Geometry check sheet. Reference: the model listing, model coordinates, mm. Face numbers are marked on the shaded views. A direction names the side the tool comes from. Round coordinates to 2 decimals unless told otherwise and drop trailing zeros. Order: outer loops, then holes, each group sorted by start corner. A loop starts at its lowest first (then second) coordinate and runs counter-clockwise, first axis right, second up. Notation, with made-up numbers: (54, 19) -> (60, 19) arc R8 ccw to (60, 31) -> close; hole circle Ø6 at (14, 44). An arc over 180 degrees is marked (long way). Use a Markdown table: item, result. Add a question column.
Item 1: Set-up check for the marked faces 1, 2, 3 and 4: record each of +Z, -Z, +X, -X, +Y, -Y from which the full face is reachable in a straight line by a thin tool's end or side.
Item 2: Sectioned sample at D-D, the plane y = 27. Record the cut outline in (x, z), and give its area (3 significant figures).
Item 3: Gauge pin test, flat ends, axial feed: pin 1 Ø5 at (y, z) = (8.5, -57) entering from -X; pin 2 Ø5 at (y, z) = (11, -56) entering from +X; pin 3 Ø10 at (x, z) = (-5, 64.5) entering from -Y. Record the tip position at first contact, or that the pin passes through.
Item 4: Sectioned sample at C-C, the plane z = 0. Record the cut outline in (x, y).
Item 5: Sectioned sample at A-A, the plane y = 7. Record the cut outline in (x, z) (1 decimal).
Item 6: Sectioned sample at B-B, the plane x = 0. Record the cut outline in (y, z).
Item 7: Mould release check, pull along Z, two halves, no side actions. Record for the marked faces 5, 6 and 7: pulls with the +Z half, pulls with the -Z half, needs draft (parallel to the pull), parting line crosses it, or undercut.
Item 8: Material ranges on probe 1 along Y at (x, z) = (-38, 44); probe 2 along Y at (x, z) = (24, 11); probe 3 along X at (y, z) = (21.25, 0), recorded low to high. Write a range as [from, to].
from build123d import *

# Parameters (mm, degrees)
BASE_DISC_20MM_DEPTH        = 20
THREE_LOBE_BOSS_15MM_DEPTH  = 15
COUNTERBORE_PROFILE_R       = 30
COUNTERBORE_20MM_DEEP_DEPTH = 20
THROUGH_BORE_PROFILE_R      = 15
THROUGH_BORE_DEPTH          = 107.05840812


with BuildPart() as part:
    # Base Disc Profile → Base Disc 20mm (new body)
    with BuildSketch(Plane(origin=(0, 0, 0), x_dir=(1, 0, 0), z_dir=(0, 1, 0))):
        with BuildLine():
            Line((-20, 53.37602458), (-20, 59.741108125))
            ThreePointArc((-20, 59.741108125), (0, 63), (20, 59.741108125))
            Line((20, 59.741108125), (20, 53.37602458))
            ThreePointArc((20, 53.37602458), (49.363448016, 28.5), (56.22499324, -9.367504214))
            Line((56.22499324, -9.367504214), (61.737317286, -12.550045987))
            ThreePointArc((61.737317286, -12.550045987), (54.559600438, -31.5), (41.737317286, -47.191062138))
            Line((41.737317286, -47.191062138), (36.22499324, -44.008520366))
            ThreePointArc((36.22499324, -44.008520366), (0, -57), (-36.22499324, -44.008520366))
            Line((-36.22499324, -44.008520366), (-41.737317286, -47.191062138))
            ThreePointArc((-41.737317286, -47.191062138), (-54.559600438, -31.5), (-61.737317286, -12.550045987))
            Line((-61.737317286, -12.550045987), (-56.22499324, -9.367504214))
            ThreePointArc((-56.22499324, -9.367504214), (-49.363448016, 28.5), (-20, 53.37602458))
        make_face()
    extrude(amount=BASE_DISC_20MM_DEPTH)

    # Three-Lobe Profile → Three-Lobe Boss 15mm (add)
    with BuildSketch(Plane(origin=(0, 20, 0), x_dir=(1, 0, 0), z_dir=(0, 1, 0))):
        with BuildLine():
            ThreePointArc((39.473039737, 41.120300752), (0, 33), (-39.473039737, 41.120300752))
            ThreePointArc((-39.473039737, 41.120300752), (-49.363448016, 28.5), (-55.347744931, 13.624504801))
            ThreePointArc((-55.347744931, 13.624504801), (-28.578838325, -16.5), (-15.874705194, -54.744805553))
            ThreePointArc((-15.874705194, -54.744805553), (-1.422355425, -56.98225079), (13.123625771, -55.468643815))
            ThreePointArc((13.123625771, -55.468643815), (27.648504036, -17.766556361), (55.906633869, 11.110728574))
            ThreePointArc((55.906633869, 11.110728574), (49.994641111, 27.377652568), (39.473039737, 41.120300752))
        make_face()
        with BuildLine():
            ThreePointArc((-39.473039737, 41.120300752), (-44.717521746, 43.555362101), (-49.812494678, 46.289473684))
            ThreePointArc((-49.812494678, 46.289473684), (-58.889727457, 34), (-64.994107477, 19.994148975))
            ThreePointArc((-64.994107477, 19.994148975), (-60.078810924, 16.948828776), (-55.347744931, 13.624504801))
            ThreePointArc((-55.347744931, 13.624504801), (-49.363448016, 28.5), (-39.473039737, 41.120300752))
        make_face()
        with BuildLine():
            ThreePointArc((-49.812494678, 46.289473684), (-52.867031225, 48.117274965), (-55.854579687, 50.052631579))
            ThreePointArc((-55.854579687, 50.052631579), (-64.951905284, 37.5), (-71.274140317, 23.345169137))
            ThreePointArc((-71.274140317, 23.345169137), (-68.104298093, 21.725554581), (-64.994107477, 19.994148975))
            ThreePointArc((-64.994107477, 19.994148975), (-58.889727457, 34), (-49.812494678, 46.289473684))
        make_face()
        with BuildLine():
            ThreePointArc((13.123625771, -55.468643815), (-1.422355425, -56.98225079), (-15.874705194, -54.744805553))
            ThreePointArc((-15.874705194, -54.744805553), (-15.361289177, -60.504190877), (-15.181612799, -66.283622659))
            ThreePointArc((-15.181612799, -66.283622659), (-1.676596285, -67.979327923), (11.895593178, -66.951436601))
            ThreePointArc((11.895593178, -66.951436601), (12.343713059, -61.192298339), (13.123625771, -55.468643815))
        make_face()
        with BuildLine():
            ThreePointArc((11.895593178, -66.951436601), (-1.676596285, -67.979327923), (-15.181612799, -66.283622659))
            ThreePointArc((-15.181612799, -66.283622659), (-15.237266868, -69.842829546), (-15.41956063, -73.397800716))
            ThreePointArc((-15.41956063, -73.397800716), (-1.839450143, -74.977439428), (11.801783935, -74.065632354))
            ThreePointArc((11.801783935, -74.065632354), (11.7853983, -70.507699919), (11.895593178, -66.951436601))
        make_face()
        with BuildLine():
            ThreePointArc((49.812494678, 46.289473684), (44.717521746, 43.555362101), (39.473039737, 41.120300752))
            ThreePointArc((39.473039737, 41.120300752), (49.994641111, 27.377652568), (55.906633869, 11.110728574))
            ThreePointArc((55.906633869, 11.110728574), (60.78874038, 14.198368606), (65.840986006, 16.998957666))
            ThreePointArc((65.840986006, 16.998957666), (59.652455781, 32.643292102), (49.812494678, 46.289473684))
        make_face()
        with BuildLine():
            ThreePointArc((55.854579687, 50.052631579), (52.867031225, 48.117274965), (49.812494678, 46.289473684))
            ThreePointArc((49.812494678, 46.289473684), (59.652455781, 32.643292102), (65.840986006, 16.998957666))
            ThreePointArc((65.840986006, 16.998957666), (69.029934048, 18.576855661), (72.272995877, 20.04031105))
            ThreePointArc((72.272995877, 20.04031105), (65.797824819, 35.995086458), (55.854579687, 50.052631579))
        make_face()
    extrude(amount=THREE_LOBE_BOSS_15MM_DEPTH)

    # Counterbore Profile → Counterbore 20mm Deep (cut)
    with BuildSketch(Plane(origin=(0, 35, 0), x_dir=(1, 0, 0), z_dir=(0, 1, 0))):
        with Locations(Location((0, 0, 0), (0, 0, 270))):
            Circle(COUNTERBORE_PROFILE_R)
    extrude(amount=-COUNTERBORE_20MM_DEEP_DEPTH, mode=Mode.SUBTRACT)

    # Through Bore Profile → Through Bore (cut, through all)
    with BuildSketch(Plane(origin=(0, 15, 0), x_dir=(1, 0, 0), z_dir=(0, 1, 0))):
        with Locations(Location((0, 0, 0), (0, 0, 270))):
            Circle(THROUGH_BORE_PROFILE_R)
    extrude(amount=-THROUGH_BORE_DEPTH, mode=Mode.SUBTRACT)


solid = part.part
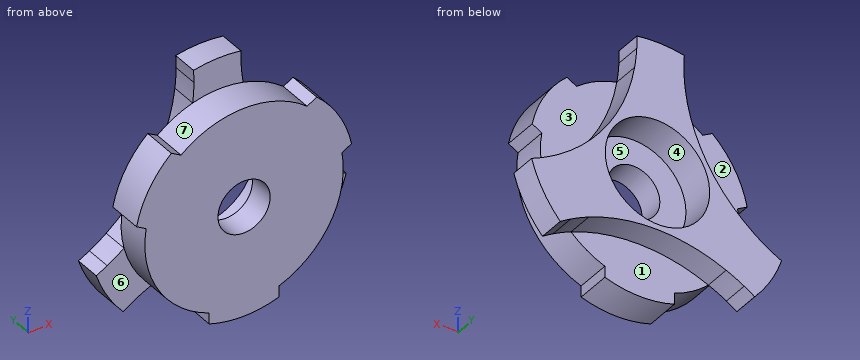
Found:
| question | item | result |
|---|---|---|
| 1 | face 1 | -Z, +Y |
| 1 | face 2 | +Z, -X, +Y |
| 1 | face 3 | +Z, +X, +Y |
| 1 | face 4 | +Y |
| 2 | outline | (-71.27, -23.35) arc R75 ccw to (-55.85, -50.05) arc R100 cw to (55.85, -50.05) arc R75 ccw to (72.27, -20.04) arc R100 cw to (11.8, 74.07) arc R75 ccw to (-15.42, 73.4) arc R100 cw to start; hole circle Ø60 at (0, 0) |
| 2 | area | 5,160 mm2 |
| 3 | pin 1 | stops at x = -20 |
| 3 | pin 2 | stops at x = 20 |
| 3 | pin 3 | stops at y = 20 |
| 4 | outline | (-57, 0) -> (-15, 0) -> (-15, 15) -> (-30, 15) -> (-30, 35) -> (-40.5, 35) -> (-40.5, 20) -> (-57, 20) -> close; (15, 0) -> (57, 0) -> (57, 20) -> (42.2, 20) -> (42.2, 35) -> (30, 35) -> (30, 15) -> (15, 15) -> close |
| 5 | outline | (-61.7, 12.6) -> (-56.2, 9.4) arc R57 ccw to (-20, -53.4) -> (-20, -59.7) arc R63 ccw to (20, -59.7) -> (20, -53.4) arc R57 ccw to (56.2, 9.4) -> (61.7, 12.6) arc R63 ccw to (41.7, 47.2) -> (36.2, 44) arc R57 ccw to (-36.2, 44) -> (-41.7, 47.2) arc R63 ccw to start; hole circle Ø30 at (0, 0) |
| 6 | outline | (0, -63) -> (20, -63) -> (20, -33) -> (35, -33) -> (35, -30) -> (15, -30) -> (15, -15) -> (0, -15) -> close; (0, 15) -> (15, 15) -> (15, 30) -> (35, 30) -> (35, 75) -> (20, 75) -> (20, 57) -> (0, 57) -> close |
| 7 | face 5 | undercut |
| 7 | face 6 | needs draft |
| 7 | face 7 | pulls with the +Z half |
| 8 | probe 1 | y = [0, 20] |
| 8 | probe 2 | y = [0, 15] |
| 8 | probe 3 | x = [-40.5, -30], [30, 42.2] |
